```python
from build123d import *

# Parameters (mm, degrees)
EXTRUDE_1_DEPTH     = 1400
CUT_EXTRUDE_1_DEPTH = 1400
SKETCH_3_R          = 30.15
CUT_EXTRUDE_2_DEPTH = 218


with BuildPart() as part:
    # 草图1 → 凸台-拉伸1 (new body)
    with BuildSketch(Plane.XY):
        with BuildLine():
            Line((-46.8, 25), (46.8, 25))
            ThreePointArc((46.8, 25), (49.0627417, 24.0627417), (50, 21.8))
            Line((50, 21.8), (50, -21.8))
            ThreePointArc((50, -21.8), (49.0627417, -24.0627417), (46.8, -25))
            Line((46.8, -25), (-46.8, -25))
            ThreePointArc((-46.8, -25), (-49.0627417, -24.0627417), (-50, -21.8))
            Line((-50, -21.8), (-50, 21.8))
            ThreePointArc((-50, 21.8), (-49.0627417, 24.0627417), (-46.8, 25))
        make_face()
        with BuildLine():
            Line((-46.8, 22), (46.8, 22))
            ThreePointArc((46.8, 22), (46.941421356, 21.941421356), (47, 21.8))
            Line((47, 21.8), (47, -21.8))
            ThreePointArc((47, -21.8), (46.941421356, -21.941421356), (46.8, -22))
            Line((46.8, -22), (-46.8, -22))
            ThreePointArc((-46.8, -22), (-46.941421356, -21.941421356), (-47, -21.8))
            Line((-47, -21.8), (-47, 21.8))
            ThreePointArc((-47, 21.8), (-46.941421356, 21.941421356), (-46.8, 22))
        make_face(mode=Mode.SUBTRACT)
    extrude(amount=EXTRUDE_1_DEPTH)

    # 草图2 → 切除-拉伸1 (cut)
    with BuildSketch(Plane(origin=(50, 0, 0), x_dir=(0, 0, -1), z_dir=(1, 0, 0))):
        Polygon((-1318.410144038, 25), (-1368.410144038, -25), (-1510.151659449, -71.563080947), (-1552.75637803, 36.507424721), align=None)
        Polygon((-54.410144038, 25), (-4.410144038, -25), (36.992690616, -46.405998122), (74.054919354, -20.164122041), (119.219041394, 25), (0, 63.525051138), align=None)
    extrude(amount=-CUT_EXTRUDE_1_DEPTH, mode=Mode.SUBTRACT)

    # 草图3 → 切除-拉伸2 (cut)
    with BuildSketch(Plane(origin=(0, 25, 0), x_dir=(1, 0, 0), z_dir=(0, 1, 0))):
        with Locations(Location((0, -686.410144038, 0), (0, 0, 270))):
            Circle(SKETCH_3_R)
    extrude(amount=-CUT_EXTRUDE_2_DEPTH, mode=Mode.SUBTRACT)


solid = part.part
```
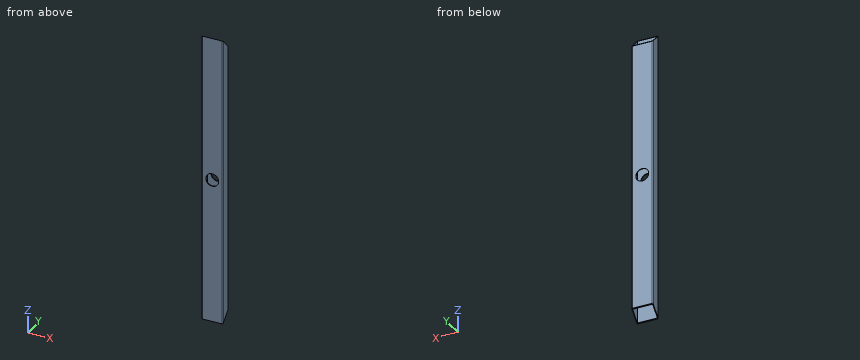
The model under review builds one solid part; all positions refer to its coordinate system, in mm. Give positions to 0.01 mm unless a question says otherwise; leave off trailing zeros. Write each loop counter-clockwise with the first axis right and the second up, starting at its lowest first coordinate (ties: lowest second). Pieces come first, ordered by that corner, then holes.
(1) Consider section B-B, the plane z = 527.5. Give the boundary of the cut face in (x, y), and give its area (3 significant figures).
(2) Consider section A-A, the plane x = 0. Give the boundary of the cut face in (y, z), and give its area (3 significant figures).
(3) To check wall thickness, follow L1, parallel to Y at x = -21.5, z = 542; L2, parallel to X at y = -9.5, z = 95.5; L3, parallel to Z at x = -18.5, y = 23.5. State the ranges of each line that lie inside material, in increasing order.
(4) Consider section C-C, the plane y = 7.5. Give the boundary of the cut face in (x, z), and give its area (3 significant figures).
Returned:
1. outline: (-50, -21.8) arc R3.2 ccw to (-46.8, -25) - (46.8, -25) arc R3.2 ccw to (50, -21.8) - (50, 21.8) arc R3.2 ccw to (46.8, 25) - (-46.8, 25) arc R3.2 ccw to (-50, 21.8) - close; hole (-47, -21.8) arc R0.2 ccw to (-46.8, -22) - (46.8, -22) arc R0.2 ccw to (47, -21.8) - (47, 21.8) arc R0.2 ccw to (46.8, 22) - (-46.8, 22) arc R0.2 ccw to (-47, 21.8) - close
1. area: 855 mm2
2. outline: (-25, 4.41) - (-22, 7.41) - (-22, 656.26) - (-25, 656.26) - close; (-25, 716.56) - (-22, 716.56) - (-22, 1365.41) - (-25, 1368.41) - close; (22, 51.41) - (25, 54.41) - (25, 656.26) - (22, 656.26) - close; (22, 716.56) - (25, 716.56) - (25, 1318.41) - (22, 1321.41) - close
2. area: 7,520 mm2
3. L1: y = -25 to -22, 22 to 25
3. L2: x = -50 to -47, 47 to 50
3. L3: z = 52.91 to 662.6, 710.22 to 1319.91
4. outline: (-50, 36.91) - (-47, 36.91) - (-47, 1335.91) - (-50, 1335.91) - close; (47, 36.91) - (50, 36.91) - (50, 1335.91) - (47, 1335.91) - close
4. area: 7,790 mm2
